from build123d import *

# Parameters (mm, degrees)
TRI_LOBE_PLATE_PROFILE_R          = 29
TRI_LOBE_PLATE_PROFILE_R_2        = 5
LOBE_PADS_EXTRUDE_20MM_DEPTH      = 10
TRI_LOBE_PLATE_PROFILE_R_3        = 4
LOBE_PADS_EXTRUDE_20MM_2_DEPTH    = 10
SKETCH1_3_R                       = 8
SKETCH1_3_R_2                     = 11
CONNECTING_WEB_EXTRUDE_14MM_DEPTH = 7


with BuildPart() as part:
    # Tri-Lobe Plate Profile → Lobe Pads Extrude 20mm (new, symmetric)
    with BuildSketch(Plane.XY):
        Circle(TRI_LOBE_PLATE_PROFILE_R)
        with Locations((-14.142135624, 14.142135624)):
            Circle(TRI_LOBE_PLATE_PROFILE_R_2, mode=Mode.SUBTRACT)
        with Locations((-20, 0)):
            Circle(TRI_LOBE_PLATE_PROFILE_R_2, mode=Mode.SUBTRACT)
        with Locations((-14.142135624, -14.142135624)):
            Circle(TRI_LOBE_PLATE_PROFILE_R_2, mode=Mode.SUBTRACT)
        with Locations((0, -20)):
            Circle(TRI_LOBE_PLATE_PROFILE_R_2, mode=Mode.SUBTRACT)
        with Locations((14.142135624, -14.142135624)):
            Circle(TRI_LOBE_PLATE_PROFILE_R_2, mode=Mode.SUBTRACT)
        with Locations((20, 0)):
            Circle(TRI_LOBE_PLATE_PROFILE_R_2, mode=Mode.SUBTRACT)
        with Locations((14.142135624, 14.142135624)):
            Circle(TRI_LOBE_PLATE_PROFILE_R_2, mode=Mode.SUBTRACT)
        with Locations((0, 20)):
            Circle(TRI_LOBE_PLATE_PROFILE_R_2, mode=Mode.SUBTRACT)
    extrude(amount=LOBE_PADS_EXTRUDE_20MM_DEPTH, both=True)



with BuildPart() as body_2:
    # Tri-Lobe Plate Profile → Lobe Pads Extrude 20mm 2 (new, symmetric)
    with BuildSketch(Plane.XY):
        with Locations((0, -68)):
            Circle(TRI_LOBE_PLATE_PROFILE_R)
        with Locations((17.320508076, -78)):
            Circle(TRI_LOBE_PLATE_PROFILE_R_3, mode=Mode.SUBTRACT)
        with Locations((17.320508076, -58)):
            Circle(TRI_LOBE_PLATE_PROFILE_R_3, mode=Mode.SUBTRACT)
        with Locations((0, -48)):
            Circle(TRI_LOBE_PLATE_PROFILE_R_3, mode=Mode.SUBTRACT)
        with Locations((-17.320508076, -58)):
            Circle(TRI_LOBE_PLATE_PROFILE_R_3, mode=Mode.SUBTRACT)
        with Locations((-17.320508076, -78)):
            Circle(TRI_LOBE_PLATE_PROFILE_R_3, mode=Mode.SUBTRACT)
        with Locations((0, -88)):
            Circle(TRI_LOBE_PLATE_PROFILE_R_3, mode=Mode.SUBTRACT)
    extrude(amount=LOBE_PADS_EXTRUDE_20MM_2_DEPTH, both=True)


with BuildPart() as part_1:
    add(part.part)

    add(body_2.part)  # Connecting Web Extrude 14mm merges body 2
    # Sketch1_3 → Connecting Web Extrude 14mm (add, symmetric)
    with BuildSketch(Plane.XY):
        with BuildLine():
            Line((-22.291841993, 18.549225875), (-55.373684133, -21.207430431))
            ThreePointArc((-55.373684133, -21.207430431), (-60, -34), (-55.373684133, -46.792569569))
            Line((-55.373684133, -46.792569569), (-22.291841993, -86.549225875))
            ThreePointArc((-22.291841993, -86.549225875), (-9.862468813, -40.728555064), (29, -68))
            ThreePointArc((29, -68), (28.999608095, -68.150765842), (28.99843239, -68.301527609))
            ThreePointArc((28.99843239, -68.301527609), (32.108419422, -59.311623745), (40, -54))
            ThreePointArc((40, -54), (59.967539964, -35.139011754), (42.274326272, -14.129734778))
            ThreePointArc((42.274326272, -14.129734778), (33.047712472, -9.497553742), (29, 0))
            ThreePointArc((29, 0), (-9.862468813, -27.271444936), (-22.291841993, 18.549225875))
        make_face()
        with Locations((-40, -34)):
            Circle(SKETCH1_3_R, mode=Mode.SUBTRACT)
        with Locations((40, -34)):
            Circle(SKETCH1_3_R_2, mode=Mode.SUBTRACT)
    extrude(amount=CONNECTING_WEB_EXTRUDE_14MM_DEPTH, both=True)


solid = part_1.part
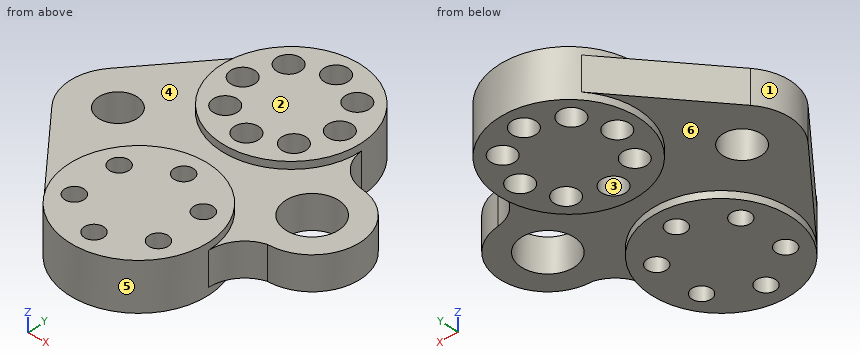
Source: CAD feature listing. Evaluate the final solid. Frame: model axes, mm. Face numbers are marked on the shaded views. A direction names the side the tool comes from. Coordinates: 2 decimals unless noted, no trailing zeros. Loops run counter-clockwise (first coordinate to the right, second up) from the corner with the lowest first, then second, coordinate; pieces in that order, holes last. Notation, with made-up numbers: (-12.75, 87) -> (2.25, 87) arc R14 ccw to (2.25, 92) -> close; hole circle Ø7 at (-20.5, 33.5). An arc over 180 degrees is marked (long way). Answer in a Markdown table with one row per item. Add a question column.
Q1. Section C-C on z = -3.5. Give the number of separate pieces and of enclosed holes in the cut face, and give its area (3 significant figures).
Q2. Ray query, line 1 along Y through (x, z) = (0, 2.25); line 2 along Y through (x, z) = (24, 8.25); line 3 along Y through (x, z) = (-13, 6.5). Return the intervals inside material, ascending.
Q3. Section D-D on y = 3. Return the cut outline in (x, z).
Q4. Section A-A on y = -88. Return the cut outline in (x, z), and give its area (3 significant figures).
Q5. Section B-B on x = 2. Return the cut outline in (y, z).
Q6. Reachability of the marked faces 4, 5 and 6 from +Z, -Z, +X, -X, +Y, -Y: full face, straight path, thin tool, end or side. Return the list, or none.
Q7. Contact query for flat-ended pins moving along their axis: pin 1 Ø5 at (x, y) = (17.32, -58) entering from -Z; pin 2 Ø16 at (x, y) = (14.14, -14.14) entering from +Z; pin 3 Ø4 at (x, z) = (-46.5, 0.5) entering from +Y; pin 4 Ø1.5 at (x, z) = (33.5, 6) entering from -Y. Output: stop coordinate, or through.
Q8. Pull-direction query (X, two-part tool) for the marked faces 1, 2 and 3; classes: pulls with the +X half, pulls with the -X half, needs draft (parallel to the pull), parting line crosses it, or undercut.
Computed values:
| question | item | result |
|---|---|---|
| 1 | separate pieces | 1 |
| 1 | enclosed holes | 16 |
| 1 | area | 7,850 mm^2 |
| 2 | line 1 | y = -97 to -92, -84 to -52, -44 to -25, -15 to 15, 25 to 29 |
| 2 | line 2 | y = -84.28 to -51.72, -16.28 to -3, 3 to 16.28 |
| 2 | line 3 | y = -93.92 to -19.01, -9.27 to 9.27, 19.01 to 25.92 |
| 3 | outline | (-35.23, -7) -> (-28.84, -7) -> (-28.84, -10) -> (-24, -10) -> (-24, 10) -> (-28.84, 10) -> (-28.84, 7) -> (-35.23, 7) -> close; (-16, -10) -> (16, -10) -> (16, 10) -> (-16, 10) -> close; (24, -10) -> (28.84, -10) -> (28.84, 10) -> (24, 10) -> close |
| 4 | outline | (-21, -10) -> (-4, -10) -> (-4, 10) -> (-21, 10) -> close; (4, -10) -> (21, -10) -> (21, 10) -> (4, 10) -> close |
| 4 | area | 680 mm^2 |
| 5 | outline | (-96.93, -10) -> (-91.46, -10) -> (-91.46, 10) -> (-96.93, 10) -> close; (-84.54, -10) -> (-51.46, -10) -> (-51.46, 10) -> (-84.54, 10) -> close; (-44.54, -10) -> (-39.07, -10) -> (-39.07, -7) -> (-28.93, -7) -> (-28.93, -10) -> (-24.58, -10) -> (-24.58, 10) -> (-28.93, 10) -> (-28.93, 7) -> (-39.07, 7) -> (-39.07, 10) -> (-44.54, 10) -> close; (-15.42, -10) -> (15.42, -10) -> (15.42, 10) -> (-15.42, 10) -> close; (24.58, -10) -> (28.93, -10) -> (28.93, 10) -> (24.58, 10) -> close |
| 6 | face 4 | +Z |
| 6 | face 5 | none |
| 6 | face 6 | -Z |
| 7 | pin 1 | passes through |
| 7 | pin 2 | stops at z = 10 |
| 7 | pin 3 | stops at y = -8.14 |
| 7 | pin 4 | stops at y = -58.53 |
| 8 | face 1 | pulls with the -X half |
| 8 | face 2 | needs draft |
| 8 | face 3 | undercut |
